from build123d import *

# Parameters (mm, degrees)
SKETCH1_W                                  = 48
SKETCH1_H                                  = 50
BOSS_EXTRUDE1_DEPTH                        = 10
SKETCH2_W                                  = 20
SKETCH2_H                                  = 20
CUT_EXTRUDE1_DEPTH                         = 10
CBORE_FOR_M6_CHEESE_HEAD_SCREW1_AT_2_COUNT = 2
CBORE_FOR_M6_CHEESE_HEAD_SCREW1_AT_2_PITCH = 22
CBORE_FOR_M6_CHEESE_HEAD_SCREW1_AT_3_COUNT = 2
CBORE_FOR_M6_CHEESE_HEAD_SCREW1_AT_3_PITCH = 38.832975678
CBORE_FOR_M6_CHEESE_HEAD_SCREW1_AT_4_COUNT = 2
CBORE_FOR_M6_CHEESE_HEAD_SCREW1_AT_4_PITCH = 32


with BuildPart() as part:
    # Sketch1 → Boss-Extrude1 (new body)
    with BuildSketch(Plane(origin=(0, 0, 0), x_dir=(1, 0, 0), z_dir=(0, 1, 0))):
        Rectangle(SKETCH1_W, SKETCH1_H)
    extrude(amount=BOSS_EXTRUDE1_DEPTH)

    # Sketch2 → Cut-Extrude1 (cut)
    with BuildSketch(Plane(origin=(0, 10, 0), x_dir=(1, 0, 0), z_dir=(0, 1, 0))):
        with Locations((0, 25)):
            Rectangle(SKETCH2_W, SKETCH2_H)
    extrude(amount=-CUT_EXTRUDE1_DEPTH, mode=Mode.SUBTRACT)

    # Sketch4 → CBORE for M6 Cheese Head Screw1 (revolve, cut)
    with BuildSketch(Plane(origin=(-16, 10, -7), x_dir=(0, 0, 1), z_dir=(1, 0, 0))):
        Polygon((0, 0), (0, 11.982840043), (3.3, 10), (3.3, 3.9), (5.5, 3.9), (5.5, 0.025), (5.525, 0), align=None)
    cbore_for_m6_cheese_head_screw1 = revolve(axis=Axis((-16, 16.35, -7), (0, -1, 0)), mode=Mode.SUBTRACT)

    # CBORE for M6 Cheese Head Screw1 at 2: CBORE for M6 Cheese Head Screw1 ×2
    with Locations(*[(0, 0, i * CBORE_FOR_M6_CHEESE_HEAD_SCREW1_AT_2_PITCH) for i in range(1, CBORE_FOR_M6_CHEESE_HEAD_SCREW1_AT_2_COUNT)]):
        add(cbore_for_m6_cheese_head_screw1, mode=Mode.SUBTRACT)

    # CBORE for M6 Cheese Head Screw1 at 3: CBORE for M6 Cheese Head Screw1 ×2
    with Locations(*[Vector(0.8240419241993677, 0, 0.5665288228870652) * (i * CBORE_FOR_M6_CHEESE_HEAD_SCREW1_AT_3_PITCH) for i in range(1, CBORE_FOR_M6_CHEESE_HEAD_SCREW1_AT_3_COUNT)]):
        add(cbore_for_m6_cheese_head_screw1, mode=Mode.SUBTRACT)

    # CBORE for M6 Cheese Head Screw1 at 4: CBORE for M6 Cheese Head Screw1 ×2
    with Locations(*[(i * CBORE_FOR_M6_CHEESE_HEAD_SCREW1_AT_4_PITCH, 0, 0) for i in range(1, CBORE_FOR_M6_CHEESE_HEAD_SCREW1_AT_4_COUNT)]):
        add(cbore_for_m6_cheese_head_screw1, mode=Mode.SUBTRACT)


solid = part.part
Geometry: final body of the model. Coordinates: model frame, mm. A direction names the side the tool comes from. Coordinates: 2 decimals unless noted, no trailing zeros. Loops run counter-clockwise (first coordinate to the right, second up) from the corner with the lowest first, then second, coordinate; pieces in that order, holes last. Notation, with made-up numbers: (46, 18) - (59, 18) arc R36 cw to (59, 52) - close; hole circle Ø2 at (49.25, 80). An arc over 180 degrees is marked (long way). One line per question, with ' | ' between items. Start each with the question number.
(1) Cut plane D-D on y = 7.75. Output: boundary loops of the cut face in (x, z), and give its area (3 significant figures).
(2) Cut plane C-C on z = 15. Output: boundary loops of the cut face in (x, y) (3 decimals).
(3) Reachability of faces 1 (the flat face through (-10, 5, -20)), 2 (the cylindrical face through (-11.1, 8.1, -4.5)), 3 (the flat face through (0, 0, 0)) from +Z, -Z, +X, -X, +Y, -Y: full face, straight path, thin tool, end or side. Return the list, or none.
(4) Cut plane A-A on y = 5.25. Output: boundary loops of the cut face in (x, z).
(5) Draft query along Z for faces 4 (the cylindrical face through (13.77, 3.09, -9.43)), 5 (the flat face through (24, 5, 0)), 6 (the flat face through (-17, 5, -25)), 7 (the flat face through (0, 5, 25)). Return one class per face: +Z half, -Z half, draft (parallel to the pull), parting line (faces both ways), or undercut.
(6) Cut plane B-B on x = 16. Output: boundary loops of the cut face in (y, z) (3 decimals), and give its area (3 significant figures).
(7) Ray query, L1, parallel to X at y = 3.5, z = 15; L2, parallel to Z at x = -16, y = 8.3; L3, parallel to Z at x = -16, y = 5.25. Return the intervals inside material, ascending. Write a range as from..to.
(8) First-contact query: pin 1 (10 mm diameter, centred on x = 16, z = -7, fed in from +Y). Flat tip, straight axial feed; report the tip coordinate or a pass-through.
Here are the results:
1) outline: (-24, -25) - (-10, -25) - (-10, -15) - (10, -15) - (10, -25) - (24, -25) - (24, 25) - (-24, 25) - close; hole circle Ø11 at (-16, -7); hole circle Ø11 at (-16, 15); hole circle Ø11 at (16, -7); hole circle Ø11 at (16, 15) | area: 1,820 mm²
2) outline: (-24, 0) - (-19.3, 0) - (-19.3, 6.1) - (-21.5, 6.1) - (-21.5, 9.975) - (-21.525, 10) - (-24, 10) - close; (-12.7, 0) - (12.7, 0) - (12.7, 6.1) - (10.5, 6.1) - (10.5, 9.975) - (10.475, 10) - (-10.475, 10) - (-10.5, 9.975) - (-10.5, 6.1) - (-12.7, 6.1) - close; (19.3, 0) - (24, 0) - (24, 10) - (21.525, 10) - (21.5, 9.975) - (21.5, 6.1) - (19.3, 6.1) - close
3) face 1: -Z, +Y, -Y | face 2: +Y | face 3: +Z, -Z, +X, -X, -Y
4) outline: (-24, -25) - (-10, -25) - (-10, -15) - (10, -15) - (10, -25) - (24, -25) - (24, 25) - (-24, 25) - close; hole circle Ø6.6 at (-16, -7); hole circle Ø6.6 at (-16, 15); hole circle Ø6.6 at (16, -7); hole circle Ø6.6 at (16, 15)
5) face 4: undercut | face 5: draft | face 6: -Z half | face 7: +Z half
6) outline: (0, -25) - (10, -25) - (10, -12.525) - (9.975, -12.5) - (6.1, -12.5) - (6.1, -10.3) - (0, -10.3) - close; (0, -3.7) - (6.1, -3.7) - (6.1, -1.5) - (9.975, -1.5) - (10, -1.475) - (10, 9.475) - (9.975, 9.5) - (6.1, 9.5) - (6.1, 11.7) - (0, 11.7) - close; (0, 18.3) - (6.1, 18.3) - (6.1, 20.5) - (9.975, 20.5) - (10, 20.525) - (10, 25) - (0, 25) - close | area: 334 mm²
7) L1: -24..-19.3, -12.7..12.7, 19.3..24 | L2: -25..-12.5, -1.5..9.5, 20.5..25 | L3: -25..-10.3, -3.7..11.7, 18.3..25
8) pin 1: y = 6.1
